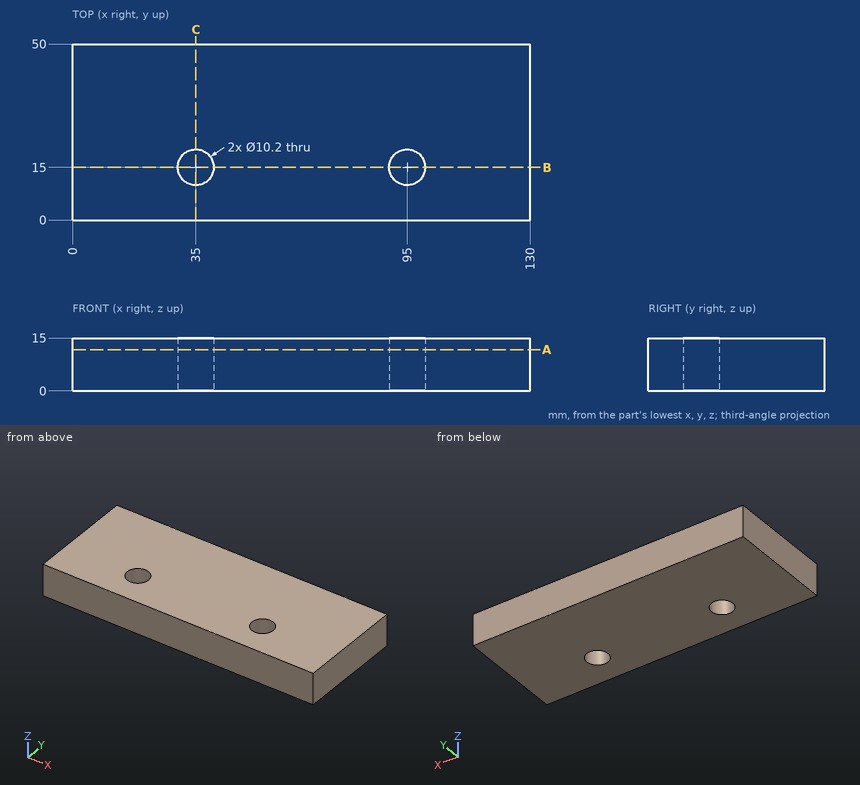
The drawing under review shows one solid part. Ordinate dimensions are in mm from its lowest x, y, z. Coordinates: 2 decimals unless noted, no trailing zeros. Write each loop counter-clockwise with the first axis right and the second up, starting at its lowest first coordinate (ties: lowest second). Pieces come first, ordered by that corner, then holes. Notation, with made-up numbers: M 62,-28 L 99,-28 A28 cw 99,-5 Z; hole C 7,18.25 d4. An arc over 180 degrees is marked long. Put each result on its own line as item: value.
1) Add section C-C on x = 35. Give the boundary of the cut face in (y, z), then the cut area to 3 significant figures.
Computed:
outline: M 0,0 L 9.9,0 L 9.9,15 L 0,15 Z; M 20.1,0 L 50,0 L 50,15 L 20.1,15 Z
area: 597 mm2
2) Wall thickness on probe 1 along Y at (x, z) = (34.5, 14.25); probe 2 along X at (y, z) = (16, 11); probe 3 along X at (y, z) = (18.5, 12.5): over which ranges is each line inside the solid? List them lowest first. Write a range as [from, to].
Computed:
probe 1: y = [0, 9.92], [20.08, 50]
probe 2: x = [0, 30], [40, 90], [100, 130]
probe 3: x = [0, 31.29], [38.71, 91.29], [98.71, 130]
3) Clearance check with a flat-ended pin moving along its axis: pin 1 Ø9 at (x, y) = (95, 15) entering from -Z. State where the tip first meets the part, or that it passes through.
Computed:
pin 1: passes through
4) Add section A-A on z = 11.75. Give the boundary of the cut face in (x, y).
Computed:
outline: M 0,0 L 130,0 L 130,50 L 0,50 Z; hole C 35,15 d10.2; hole C 95,15 d10.2
5) Add section B-B on y = 15. Give the boundary of the cut face in (x, z), then the cut area to 3 significant figures.
Computed:
outline: M 0,0 L 29.9,0 L 29.9,15 L 0,15 Z; M 40.1,0 L 89.9,0 L 89.9,15 L 40.1,15 Z; M 100.1,0 L 130,0 L 130,15 L 100.1,15 Z
area: 1,640 mm2
